Geometry check sheet. Reference: the model listing, model coordinates, mm. A direction names the side the tool comes from. Round coordinates to 2 decimals unless told otherwise and drop trailing zeros. Loops run counter-clockwise (first coordinate to the right, second up) from the corner with the lowest first, then second, coordinate; pieces in that order, holes last. Notation, with made-up numbers: (22.5, 63.25) -> (67.5, 63.25) arc R32 cw to (67.5, 97.25) -> close; hole circle Ø5 at (-10.5, -29). An arc over 180 degrees is marked (long way). Use one line per item in the form item = value.
from build123d import *

# Parameters (mm, degrees)
BOSS_EXTRUDE1_DEPTH = 300


with BuildPart() as part:
    # Sketch1 → Boss-Extrude1 (new body)
    with BuildSketch(Plane(origin=(0, 0, 0), x_dir=(1, 0, 0), z_dir=(0, 1, 0))):
        Polygon((0, 23.094010768), (-20, 11.547005384), (-20, -11.547005384), (0, -23.094010768), (20, -11.547005384), (20, 11.547005384), align=None)
        Polygon((-17, 9.814954576), (-17, -9.814954576), (0, -19.629909152), (17, -9.814954576), (17, 9.814954576), (0, 19.629909152), align=None, mode=Mode.SUBTRACT)
    extrude(amount=BOSS_EXTRUDE1_DEPTH)


solid = part.part
1. Tool access check on faces 1 (the flat face through (8.619, 147.9, -14.654)), 2 (the flat face through (-9, 300, 15)). Record the directions out of +Z, -Z, +X, -X, +Y, -Y that give a thin tool (end or side, any length) a straight path to the whole face; none if there is none.
Return value:
face_1 = +Y, -Y
face_2 = +Z, -Z, +X, -X, +Y
2. Material ranges on line 1 along X through (y, z) = (32, -3); line 2 along Z through (x, y) = (-10, 250); line 3 along X through (y, z) = (256.5, 19), recorded low to high.
Return value:
line_1 = -20 to -17, 17 to 20
line_2 = -17.32 to -13.86, 13.86 to 17.32
line_3 = -7.09 to -1.09, 1.09 to 7.09
3. Mould release check, pull along Z, two halves, no side actions. Record for faces 3 (the flat face through (-9.86, 147.9, -17.4)), 4 (the flat face through (-17, 148, 0)), 5 (the flat face through (-10.14, 147.9, 17.24)): released by +Z, released by -Z, zero draft, split by the parting line, or undercut.
Return value:
face_3 = released by -Z
face_4 = undercut
face_5 = released by +Z
4. Section check B-B (y = 109.5). Record the boundary of the cut face in (x, z), then the cut area to 3 significant figures.
Return value:
outline = (-20, -11.55) -> (0, -23.09) -> (20, -11.55) -> (20, 11.55) -> (0, 23.09) -> (-20, 11.55) -> close; hole (-17, -9.81) -> (0, -19.63) -> (17, -9.81) -> (17, 9.81) -> (0, 19.63) -> (-17, 9.81) -> close
area = 385 mm2
5. Section check A-A (z = 2). Record the boundary of the cut face in (x, y).
Return value:
outline = (-20, 0) -> (-17, 0) -> (-17, 300) -> (-20, 300) -> close; (17, 0) -> (20, 0) -> (20, 300) -> (17, 300) -> close
6. Gauge pin test, flat ends, axial feed: pin 1 (12 mm diameter, centred on x = 6.5, y = 142, fed in from +Z); pin 2 (2 mm diameter, centred on y = 138.5, z = 13, fed in from +X). Record the tip position at first contact, or that the pin passes through.
Return value:
pin_1 = 22.81
pin_2 = 19.22
7. Section check C-C (x = 3.5). Record the boundary of the cut face in (y, z).
Return value:
outline = (0, -21.07) -> (300, -21.07) -> (300, -17.61) -> (0, -17.61) -> close; (0, 17.61) -> (300, 17.61) -> (300, 21.07) -> (0, 21.07) -> close
